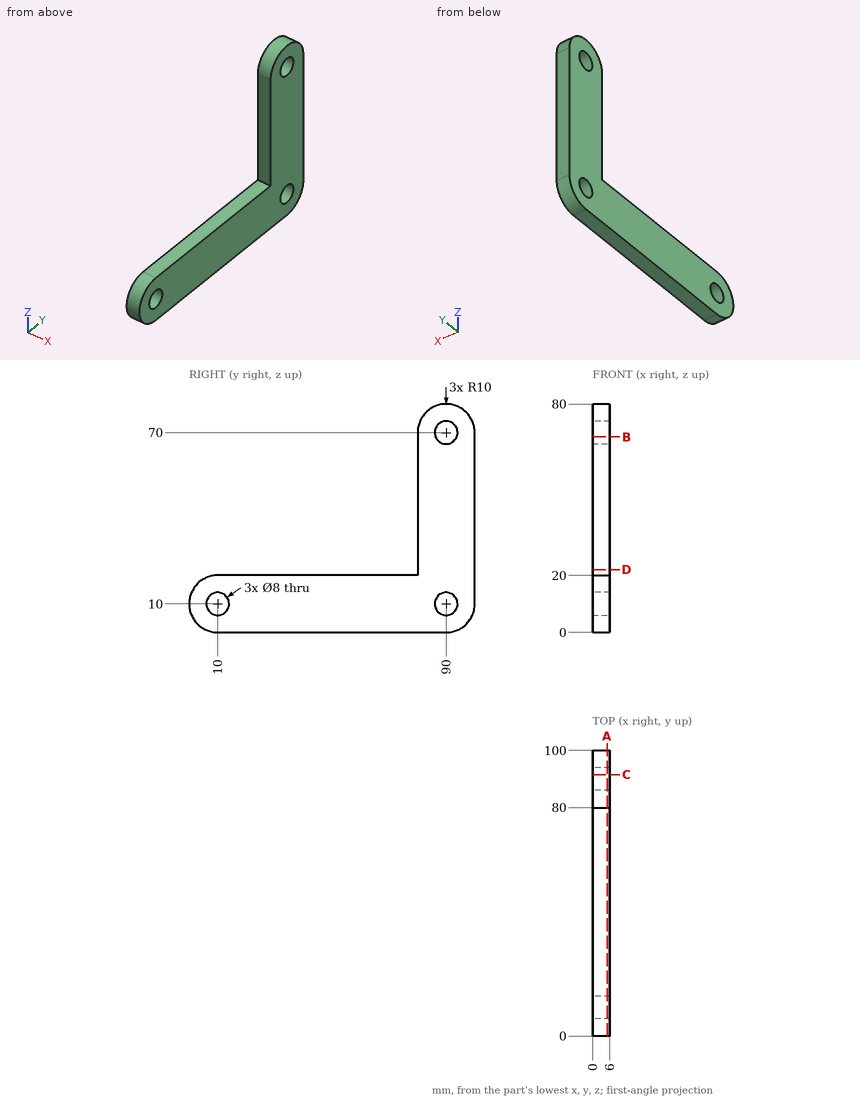
Geometry check sheet. Reference: drawing and pictorial views, mm from the part's lowest x, y, z. Coordinates: 2 decimals unless noted, no trailing zeros. Order: outer loops, then holes, each group sorted by start corner. A loop starts at its lowest first (then second) coordinate and runs counter-clockwise, first axis right, second up. Notation, with made-up numbers: (87, 72.5) -> (112, 72.5) arc R31 ccw to (112, 104.5) -> close; hole circle Ø1 at (-10, 69.5). An arc over 180 degrees is marked (long way). Write item = value, one per line. Start each with the question number.
1) Cross-section at C-C (y = 91.5). Enter the section's corners in (x, z), then the cut area to 3 significant figures.
2) Cross-section at B-B (z = 68.5). Enter the section's corners in (x, y).
3) Go/stop test with flat-tipped pins: P1, Ø6.5, axis at y = 90, z = 10, coming from the +X side; P2, Ø3, axis at x = 3.5, y = 51.5, coming from the +Z side. Record where each tip stops, or that it passes through.
4) Material ranges on L1, parallel to Y at x = 1.9, z = 10; L2, parallel to Y at x = 3.4, z = 70; L3, parallel to Y at x = 0.65, z = 73, recorded low to high.
5) Cross-section at D-D (z = 22). Enter the section's corners in (x, y).
6) Cross-section at A-A (x = 5.05). Enter the section's corners in (y, z).
Ans:
q1.outline = (0, 0.11) -> (6, 0.11) -> (6, 6.29) -> (0, 6.29) -> close; (0, 13.71) -> (6, 13.71) -> (6, 66.29) -> (0, 66.29) -> close; (0, 73.71) -> (6, 73.71) -> (6, 79.89) -> (0, 79.89) -> close
q1.area = 390 mm²
q2.outline = (0, 80) -> (6, 80) -> (6, 86.29) -> (0, 86.29) -> close; (0, 93.71) -> (6, 93.71) -> (6, 100) -> (0, 100) -> close
q3.P1 = through
q3.P2 = 20
q4.L1 = 0 to 6, 14 to 86, 94 to 100
q4.L2 = 80 to 86, 94 to 100
q4.L3 = 80.46 to 87.35, 92.65 to 99.54
q5.outline = (0, 80) -> (6, 80) -> (6, 100) -> (0, 100) -> close
q6.outline = (10, 0) -> (90, 0) arc R10 ccw to (100, 10) -> (100, 70) arc R10 ccw to (80, 70) -> (80, 20) -> (10, 20) arc R10 ccw to start; hole circle Ø8 at (10, 10); hole circle Ø8 at (90, 10); hole circle Ø8 at (90, 70)
